```python
from build123d import *

# Parameters (mm, degrees)
BOSS_EXTRUDE1_DEPTH = 8.4
SKETCH5_R           = 5
CUT_EXTRUDE1_DEPTH  = 15.828800806


with BuildPart() as part:
    # Sketch1 → Boss-Extrude1 (new body)
    with BuildSketch(Plane.XY):
        Polygon((0, 9.237604307), (-8, 4.618802154), (-8, -4.618802154), (0, -9.237604307), (8, -4.618802154), (8, 4.618802154), align=None)
    extrude(amount=BOSS_EXTRUDE1_DEPTH)

    # Sketch4 → Cut-Revolve1 (revolve, cut)
    with BuildSketch(Plane(origin=(0, 0, 0), x_dir=(0, 0, -1), z_dir=(1, 0, 0)), mode=Mode.PRIVATE) as cut_revolve1_sk:
        Polygon((-8.4, -7.2), (-7.658372683, -9.237604307), (-8.4, -9.237604307), align=None)
    cut_revolve1 = revolve(cut_revolve1_sk.sketch.rotate(Axis((0, 0, 8.4), (0, 0, -1)), 119.999999987), axis=Axis((0, 0, 8.4), (0, 0, -1)), mode=Mode.SUBTRACT)

    # Mirror1: Cut-Revolve1 across plane
    add(cut_revolve1.mirror(Plane.XY.offset(4.2)), mode=Mode.SUBTRACT)

    # Sketch5 → Cut-Extrude1 (cut, through all)
    with BuildSketch(Plane.XY.offset(8.4)):
        Circle(SKETCH5_R)
    extrude(amount=-CUT_EXTRUDE1_DEPTH, mode=Mode.SUBTRACT)


solid = part.part
```
Part model, mm, in its own coordinate system. Round coordinates to 2 decimals unless told otherwise and drop trailing zeros. Loops run counter-clockwise (first coordinate to the right, second up) from the corner with the lowest first, then second, coordinate; pieces in that order, holes last.
Item 1: Mould opens along Y. For faces 1 (the face through (-2, 5, 0)), 2 (the face through (-1.08, -4.88, 4.26)), 3 (the face through (4.056, 6.896, 4.145)) say: +Y half, -Y half, draft (parallel to the pull), parting line (faces both ways), or undercut.
Item 2: Cut at A-A, the plane y = 0. Give the cut face in (x, z), then the cut area to 3 significant figures.
Item 3: Drill centre lines: line 1 (X direction, y = -0.25, z = 5.75); line 2 (Y direction, x = 3.5, z = 1); line 3 (Y direction, x = -1.5, z = 7). Where is each one in solid material? Low to high.
A:
1. face 1: draft
1. face 2: undercut
1. face 3: +Y half
2. outline: (-8, 0.29) - (-7.2, 0) - (-5, 0) - (-5, 8.4) - (-7.2, 8.4) - (-8, 8.11) - close; (5, 0) - (7.2, 0) - (8, 0.29) - (8, 8.11) - (7.2, 8.4) - (5, 8.4) - close
2. area: 49.9 mm2
3. line 1: x = -8 to -4.99, 4.99 to 8
3. line 2: y = -7.22 to -3.57, 3.57 to 7.22
3. line 3: y = -8.37 to -4.77, 4.77 to 8.37
